```python
from build123d import *

# Parameters (mm, degrees)
SKETCH1_W           = 40
SKETCH1_H           = 40
BOSS_EXTRUDE1_DEPTH = 25
SKETCH2_W           = 40
SKETCH2_H           = 30
CUT_EXTRUDE1_DEPTH  = 10
M6_TAPPED_HOLE1_D   = 5


with BuildPart() as part:
    # Sketch1 → Boss-Extrude1 (new body)
    with BuildSketch(Plane(origin=(0, 0, 0), x_dir=(1, 0, 0), z_dir=(0, 1, 0))):
        Rectangle(SKETCH1_W, SKETCH1_H)
    extrude(amount=BOSS_EXTRUDE1_DEPTH)

    # Sketch2 → Cut-Extrude1 (cut)
    with BuildSketch(Plane(origin=(0, 25, 0), x_dir=(1, 0, 0), z_dir=(0, 1, 0))):
        Rectangle(SKETCH2_W, SKETCH2_H)
    extrude(amount=-CUT_EXTRUDE1_DEPTH, mode=Mode.SUBTRACT)

    # M6 Tapped Hole1 (through all)
    with Locations(Plane(origin=(0, 0, 0), x_dir=(-1, 0, 0), z_dir=(0, -1, 0))):
        with Locations((0, 0)):
            Hole(M6_TAPPED_HOLE1_D / 2)


solid = part.part
```
Geometry: final body of the model. Coordinates: model frame, mm. A direction names the side the tool comes from. Coordinates: 2 decimals unless noted, no trailing zeros. Loops run counter-clockwise (first coordinate to the right, second up) from the corner with the lowest first, then second, coordinate; pieces in that order, holes last. Notation, with made-up numbers: (-36, -21.75) -> (-3, -21.75) arc R27 ccw to (-3, 10.25) -> close; hole circle Ø7 at (-18.75, 17). An arc over 180 degrees is marked (long way). Use a Markdown table: item, result. Add a question column.
(1) Section query C-C, the plane y = 23. Return loops of the section in (x, z), plus the area to 3 significant figures.
(2) Section query A-A, the plane z = 0. Return loops of the section in (x, y).
(3) Line query: line 1 along Z through (x, y) = (0, 8); line 2 along Z through (x, y) = (1, 17.25); line 3 along Y through (x, z) = (-16, -2). Output: solid intervals per line, ascending.
(4) Section query D-D, the plane x = 4. Return loops of the section in (y, z).
(5) Mould query, pull axis Z, two halves, no side actions, for faces 1 (the flat face through (0, 12, 20)), 2 (the cylindrical face through (-0.54, 7.6, 2.44)), 3 (the flat face through (0, 25, 17)). Classes: pulls with the +Z half, pulls with the -Z half, needs draft (parallel to the pull), parting line crosses it, or undercut.
(6) Access query for faces 4 (the flat face through (0, 15, -4)), 5 (the flat face through (0, 12, -20)). Directions: +Z, -Z, +X, -X, +Y, -Y. A direction counts if a zero-diameter tool reaches every point of the face in a straight line with its end or side. Return the directions, or none.
(7) Section query B-B, the plane x = 0. Return loops of the section in (y, z), plus the area to 3 significant figures.
Answer:
| question | item | result |
|---|---|---|
| 1 | outline | (-20, -20) -> (20, -20) -> (20, -15) -> (-20, -15) -> close; (-20, 15) -> (20, 15) -> (20, 20) -> (-20, 20) -> close |
| 1 | area | 400 mm^2 |
| 2 | outline | (-20, 0) -> (-2.5, 0) -> (-2.5, 15) -> (-20, 15) -> close; (2.5, 0) -> (20, 0) -> (20, 15) -> (2.5, 15) -> close |
| 3 | line 1 | z = -20 to -2.5, 2.5 to 20 |
| 3 | line 2 | z = -20 to -15, 15 to 20 |
| 3 | line 3 | y = 0 to 15 |
| 4 | outline | (0, -20) -> (25, -20) -> (25, -15) -> (15, -15) -> (15, 15) -> (25, 15) -> (25, 20) -> (0, 20) -> close |
| 5 | face 1 | pulls with the +Z half |
| 5 | face 2 | undercut |
| 5 | face 3 | needs draft |
| 6 | face 4 | +X, -X, +Y |
| 6 | face 5 | -Z, +X, -X, +Y, -Y |
| 7 | outline | (0, -20) -> (25, -20) -> (25, -15) -> (15, -15) -> (15, -2.5) -> (0, -2.5) -> close; (0, 2.5) -> (15, 2.5) -> (15, 15) -> (25, 15) -> (25, 20) -> (0, 20) -> close |
| 7 | area | 625 mm^2 |
